The drawing under review shows one solid part. Ordinate dimensions are in mm from its lowest x, y, z. Coordinates: 2 decimals unless noted, no trailing zeros. Loops run counter-clockwise (first coordinate to the right, second up) from the corner with the lowest first, then second, coordinate; pieces in that order, holes last. Notation, with made-up numbers: (22, 63.5) -> (52, 63.5) arc R30 cw to (52, 86.5) -> close; hole circle Ø2 at (28.25, 41). An arc over 180 degrees is marked (long way). Use a Markdown table: item, result.
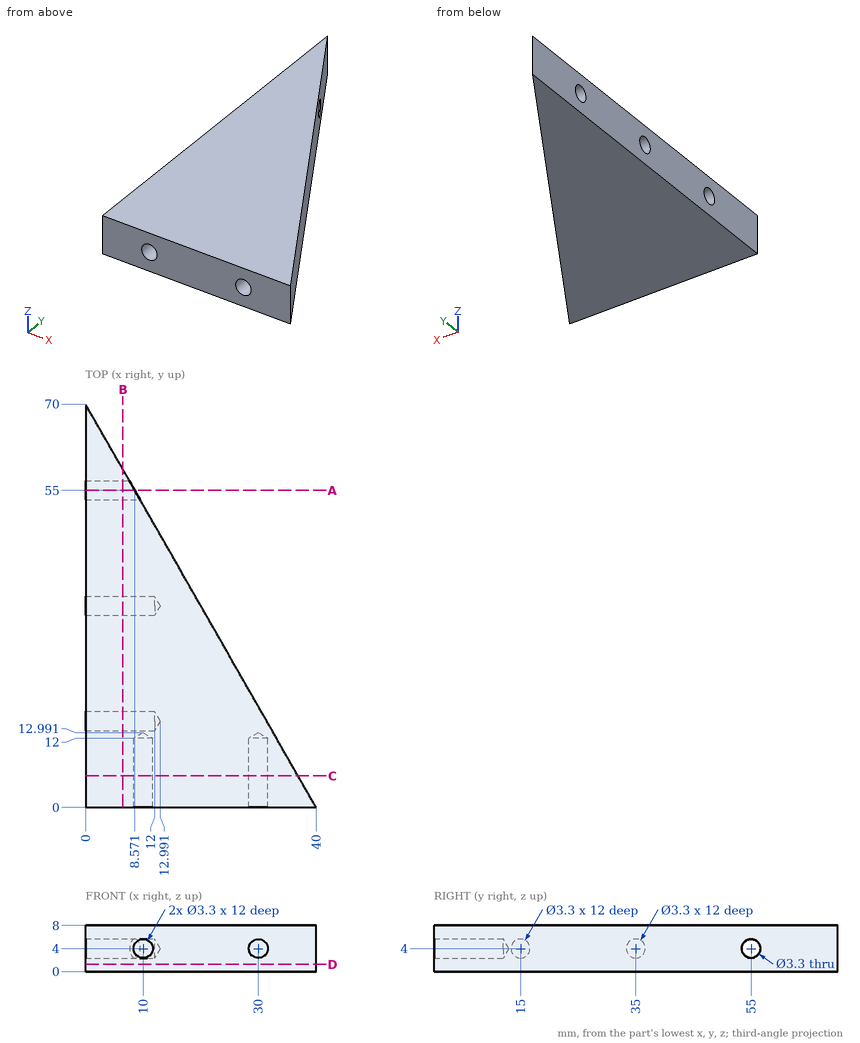
(1) Take a section at D-D on z = 1.25. Write out the cut boundary in (x, y).
Found:
| item | result |
|---|---|
| outline | (0, 0) -> (40, 0) -> (0, 70) -> close |
(2) Take a section at B-B on x = 6.5. State how many separate pieces and enclosed holes the cut face has, plus the area to 3 significant figures.
Found:
| item | result |
|---|---|
| separate pieces | 1 |
| enclosed holes | 3 |
| area | 443 mm^2 |
(3) Take a section at C-C on y = 5.5. Write out the cut boundary in (x, z), plus the area to 3 significant figures.
Found:
| item | result |
|---|---|
| outline | (0, 0) -> (36.86, 0) -> (36.86, 8) -> (0, 8) -> close; hole circle Ø3.3 at (10, 4); hole circle Ø3.3 at (30, 4) |
| area | 278 mm^2 |
(4) For pin 1 Ø2 at (x, y) = (4, 56) entering from -Z; pin 2 Ø2.5 at (y, z) = (35, 4) entering from -X; pin 3 Ø4 at (y, z) = (31.5, 4.5) entering from +X; pin 4 Ø3 at (y, z) = (15, 4) entering from +X (1 decimal), all flat-tipped, find the tip position at first contact; note any pin that passes through.
Found:
| item | result |
|---|---|
| pin 1 | stops at z = 0 |
| pin 2 | stops at x = 12.24 |
| pin 3 | stops at x = 23.14 |
| pin 4 | stops at x = 32.3 |
(5) For line 1 along Z through (x, y) = (30, 3); line 2 along Y through (x, z) = (6, 4); line 3 along Y through (x, z) = (11, 4), list the stretches that pass through material, from the lowest coordinate up.
Found:
| item | result |
|---|---|
| line 1 | z = 0 to 2.35, 5.65 to 8 |
| line 2 | y = 0 to 13.35, 16.65 to 33.35, 36.65 to 53.35, 56.65 to 59.5 |
| line 3 | y = 12.39 to 13.35, 16.65 to 33.35, 36.65 to 50.75 |
(6) Take a section at A-A on y = 55. Write out the cut boundary in (x, z).
Found:
| item | result |
|---|---|
| outline | (0, 0) -> (8.57, 0) -> (8.57, 2.35) -> (0, 2.35) -> close; (0, 5.65) -> (8.57, 5.65) -> (8.57, 8) -> (0, 8) -> close |
